```python
from build123d import *

# Parameters (mm, degrees)
SKETCH1_R           = 12.6
BOSS_EXTRUDE1_DEPTH = 10.8
SKETCH2_W           = 36
SKETCH2_H           = 36
BOSS_EXTRUDE2_DEPTH = 7.2
FILLET1_R           = 3.6
CHAMFER1_SIZE       = 0.72
SKETCH3_R           = 14.4
SKETCH3_R_2         = 12.6
CUT_EXTRUDE1_DEPTH  = 1.08
SKETCH4_W           = 1.08
SKETCH4_H           = 0.54
SKETCH5_R           = 1.62
CUT_EXTRUDE2_DEPTH  = 7.2
SKETCH6_R           = 8.1
CUT_EXTRUDE3_DEPTH  = 10.8


with BuildPart() as part:
    # Sketch1 → Boss-Extrude1 (new body)
    with BuildSketch(Plane.XY):
        with Locations(Location((0, 0, 0), (0, 0, 180))):
            Circle(SKETCH1_R)
    extrude(amount=BOSS_EXTRUDE1_DEPTH)

    # Sketch2 → Boss-Extrude2 (add)
    with BuildSketch(Plane.XY.offset(10.8)):
        Rectangle(SKETCH2_W, SKETCH2_H)
    extrude(amount=BOSS_EXTRUDE2_DEPTH)

    # Fillet1
    fillet1_edges = [part.edges().sort_by_distance(p)[0] for p in [
        (18, -18, 14.4),
        (18, 18, 14.4),
        (-18, 18, 14.4),
        (-18, -18, 14.4),
    ]]
    fillet(fillet1_edges, radius=FILLET1_R)

    # Chamfer1
    chamfer1_edges = [part.edges().sort_by_distance(p)[0] for p in [
        (12.6, 0, 0),
    ]]
    chamfer(chamfer1_edges, length=CHAMFER1_SIZE)

    # Sketch3 → Cut-Extrude1 (cut)
    with BuildSketch(Plane(origin=(0, 0, 10.8), x_dir=(-1, 0, 0), z_dir=(0, 0, -1))):
        Circle(SKETCH3_R)
        Circle(SKETCH3_R_2, mode=Mode.SUBTRACT)
    extrude(amount=-CUT_EXTRUDE1_DEPTH, mode=Mode.SUBTRACT)

    # Sketch4 → Cut-Revolve1 (revolve, cut)
    with BuildSketch(Plane(origin=(0, 0, 0), x_dir=(1, 0, 0), z_dir=(0, 1, 0)), mode=Mode.PRIVATE) as cut_revolve1_sk:
        with Locations((12.6, -6.3)):
            Rectangle(SKETCH4_W, SKETCH4_H)
    revolve(cut_revolve1_sk.sketch.rotate(Axis((0, 0, -2.746665179), (0, 0, 1)), 180), axis=Axis((0, 0, -2.746665179), (0, 0, 1)), mode=Mode.SUBTRACT)

    # Sketch5 → Cut-Extrude2 (cut)
    with BuildSketch(Plane(origin=(0, 0, 10.8), x_dir=(-1, 0, 0), z_dir=(0, 0, -1))):
        with Locations((14.4, 14.4)):
            Circle(SKETCH5_R)
        with Locations((14.4, -14.4)):
            Circle(SKETCH5_R)
        with Locations((-14.4, -14.4)):
            Circle(SKETCH5_R)
        with Locations((-14.4, 14.4)):
            Circle(SKETCH5_R)
    extrude(amount=-CUT_EXTRUDE2_DEPTH, mode=Mode.SUBTRACT)

    # Sketch6 → Cut-Extrude3 (cut)
    with BuildSketch(Plane(origin=(0, 0, 0), x_dir=(-1, 0, 0), z_dir=(0, 0, -1))):
        Circle(SKETCH6_R)
    extrude(amount=-CUT_EXTRUDE3_DEPTH, mode=Mode.SUBTRACT)


solid = part.part
```
CAD build for the part. Positions are in the model's coordinates, mm. A direction names the side the tool comes from. Round coordinates to 2 decimals unless told otherwise and drop trailing zeros. Write each loop counter-clockwise with the first axis right and the second up, starting at its lowest first coordinate (ties: lowest second). Pieces come first, ordered by that corner, then holes. Notation, with made-up numbers: (55, -32) - (111, -32) arc R16 ccw to (111, -28) - close; hole circle Ø11 at (8.5, 25.5). An arc over 180 degrees is marked (long way). Write item = value, one per line. Start each with the question number.
Q1. Which spindle directions (+Z, -Z, +X, -X, +Y, -Y) get a long thin tool onto all of the face, cutting with end or side? Do faces 1 (the cylindrical face through (-15.271, 15.766, 14.35)), 2 (the cylindrical face through (-13.735, 4.325, 11.332)). Say none if no direction does.
Q2. Band-saw the part on D-D (z = 4.75). Give the cut face in (x, y), then the cut area to 3 significant figures.
Q3. Probe L1, parallel to Y at x = 14.4, z = 15.25; L2, parallel to Y at x = 0, z = 11.3; L3, parallel to X at y = 5, z = 11.25. List the from-to ranges inside material, lowest first. Write a range as from..to.
Q4. Mould opens along Y. For faces 3 (the flat face through (0, 18, 14)), 4 (the flat face through (0, 0, 10.8)), 5 (the flat face through (-8, -3, 0)) say: pulls with the +Y half, pulls with the -Y half, needs draft (parallel to the pull), parting line crosses it, or undercut.
Q5. Band-saw the part on A-A (z = 13.75). Give the cut face in (x, y).
Q6. Band-saw the part on B-B (y = 0). Give the cut face in (x, z).
Q7. Drop flat-ended pins along their axis: pin 1 (8 mm diameter, centred on x = -3.5, y = 1, fed in from -Z); pin 2 (10 mm diameter, centred on y = 11, z = 2.5, fed in from +X); pin 3 (1 mm diameter, centred on x = 9, z = 2.5, fed in from -Y). Give the stop position or say it passes through.
Answers below:
q1.face_1 = +Z, -Z
q1.face_2 = -Z
q2.outline = circle Ø25.2 at (0, 0); hole circle Ø16.2 at (0, 0)
q2.area = 293 mm2
q3.L1 = -18..-16.02, -12.78..12.78, 16.02..18
q3.L2 = -18..-14.4, -12.6..12.6, 14.4..18
q3.L3 = -18..-13.5, -11.57..11.57, 13.5..18
q4.face_3 = pulls with the +Y half
q4.face_4 = undercut
q4.face_5 = needs draft
q5.outline = (-18, -14.4) arc R3.6 ccw to (-14.4, -18) - (14.4, -18) arc R3.6 ccw to (18, -14.4) - (18, 14.4) arc R3.6 ccw to (14.4, 18) - (-14.4, 18) arc R3.6 ccw to (-18, 14.4) - close; hole circle Ø3.24 at (-14.4, -14.4); hole circle Ø3.24 at (-14.4, 14.4); hole circle Ø3.24 at (14.4, -14.4); hole circle Ø3.24 at (14.4, 14.4)
q6.outline = (-18, 10.8) - (-14.4, 10.8) - (-14.4, 11.88) - (-12.6, 11.88) - (-12.6, 6.57) - (-12.06, 6.57) - (-12.06, 6.03) - (-12.6, 6.03) - (-12.6, 0.72) - (-11.88, 0) - (-8.1, 0) - (-8.1, 10.8) - (8.1, 10.8) - (8.1, 0) - (11.88, 0) - (12.6, 0.72) - (12.6, 6.03) - (12.06, 6.03) - (12.06, 6.57) - (12.6, 6.57) - (12.6, 11.88) - (14.4, 11.88) - (14.4, 10.8) - (18, 10.8) - (18, 18) - (-18, 18) - close
q7.pin_1 = 10.8
q7.pin_2 = 11.08
q7.pin_3 = -9.3
